Job drawing, mm, ordinate dimensions from the low corner. One solid piece. A direction names the side the tool comes from. Give positions to 0.01 mm unless a question says otherwise; leave off trailing zeros. Order: outer loops, then holes, each group sorted by start corner. A loop starts at its lowest first (then second) coordinate and runs counter-clockwise, first axis right, second up.
1. Probe line 1 (Y direction, x = 110, z = 21); line 2 (X direction, y = 7.5, z = 13.5); line 3 (X direction, y = 28, z = 15). List the from-to ranges inside material, lowest first.
2. Slice it at A-A on y = 33. List the corners of the cut face in (x, z).
3. Slice it at C-C on x = 15. List the corners of the cut face in (y, z).
4. Slice it at B-B on x = 110. List the corners of the cut face in (y, z).
5. Mould opens along Z. For the marked faces 4, 5 and 6 say: +Z half, -Z half, draft (parallel to the pull), parting line (faces both ways), or undercut.
6. Which spindle directions (+Z, -Z, +X, -X, +Y, -Y) get a long thin tool onto all of the face, cutting with end or side? Do the marked faces 1, 2 and 3. Say none if no direction does.
7. Slice it at D-D on z = 32.5. List the corners of the cut face in (x, y), and give its area (3 significant figures).
8. Drop a flat-ended pin along its axis: pin 1 Ø4 at (y, z) = (43, 53) entering from +X. Give the stop position or say it passes through.
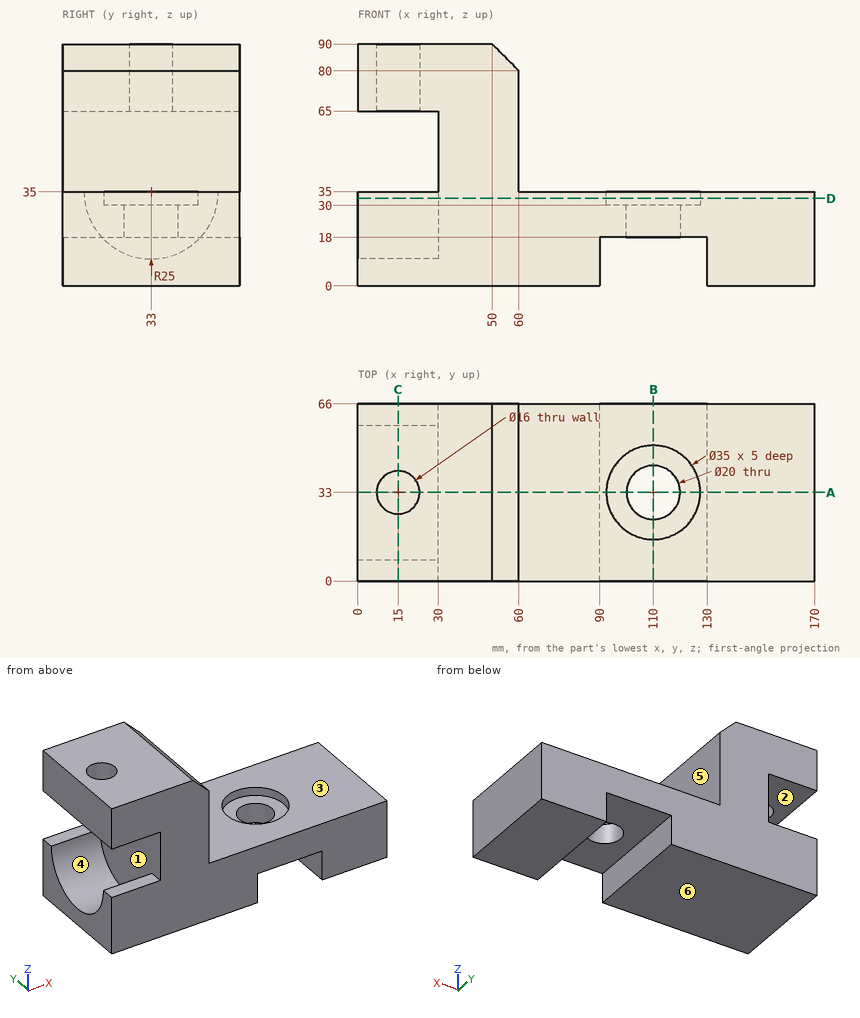
Data:
1. line 1: y = 0 to 23, 43 to 66
1. line 2: x = 0 to 90, 130 to 170
1. line 3: x = 30 to 90, 130 to 170
2. outline: (0, 0) - (90, 0) - (90, 18) - (100, 18) - (100, 30) - (92.5, 30) - (92.5, 35) - (60, 35) - (60, 80) - (50, 90) - (23, 90) - (23, 65) - (30, 65) - (30, 10) - (0, 10) - close; (0, 65) - (7, 65) - (7, 90) - (0, 90) - close; (120, 18) - (130, 18) - (130, 0) - (170, 0) - (170, 35) - (127.5, 35) - (127.5, 30) - (120, 30) - close
3. outline: (0, 0) - (66, 0) - (66, 35) - (58, 35) arc R25 cw to (8, 35) - (0, 35) - close; (0, 65) - (25, 65) - (25, 90) - (0, 90) - close; (41, 65) - (66, 65) - (66, 90) - (41, 90) - close
4. outline: (0, 18) - (23, 18) - (23, 30) - (15.5, 30) - (15.5, 35) - (0, 35) - close; (43, 18) - (66, 18) - (66, 35) - (50.5, 35) - (50.5, 30) - (43, 30) - close
5. face 4: undercut
5. face 5: draft
5. face 6: -Z half
6. face 1: -X
6. face 2: -X, +Y, -Y
6. face 3: +Z, +X, +Y, -Y
7. outline: (0, 0) - (170, 0) - (170, 66) - (0, 66) - (0, 57.87) - (30, 57.87) - (30, 8.13) - (0, 8.13) - close; hole circle Ø35 at (110, 33)
7. area: 8,770 mm2
8. pin 1: stops at x = 60
